from build123d import *

# Parameters (mm, degrees)
BOSS_EXTRUDE1_DEPTH        = 8
F_11_0_11_DIAMETER_HOLE5_D = 11


with BuildPart() as part:
    # Sketch1 → Boss-Extrude1 (new body)
    with BuildSketch(Plane.XY):
        with BuildLine():
            Line((20, -75), (-20, -75))
            ThreePointArc((-20, -75), (-23.535533906, -73.535533906), (-25, -70))
            Line((-25, -70), (-25, 70))
            ThreePointArc((-25, 70), (-23.535533906, 73.535533906), (-20, 75))
            Line((-20, 75), (20, 75))
            ThreePointArc((20, 75), (23.535533906, 73.535533906), (25, 70))
            Line((25, 70), (25, -70))
            ThreePointArc((25, -70), (23.535533906, -73.535533906), (20, -75))
        make_face()
    extrude(amount=BOSS_EXTRUDE1_DEPTH)

    # Ø11.0 (11) Diameter Hole5 (through all)
    with Locations(Plane.XY.offset(8)):
        with Locations((0, 52.5), (0, -52.5)):
            Hole(F_11_0_11_DIAMETER_HOLE5_D / 2)


solid = part.part
Here's how the part is built. I have some questions about the finished solid (model axes, mm). Coordinates: 2 decimals unless noted, no trailing zeros. Order: outer loops, then holes, each group sorted by start corner. A loop starts at its lowest first (then second) coordinate and runs counter-clockwise, first axis right, second up.
Item 1: If we section it at C-C on z = 2.25: List the corners of the cut face in (x, y) for me.
Result sheet:
outline: (-25, -70) arc R5 ccw to (-20, -75) - (20, -75) arc R5 ccw to (25, -70) - (25, 70) arc R5 ccw to (20, 75) - (-20, 75) arc R5 ccw to (-25, 70) - close; hole circle Ø11 at (0, -52.5); hole circle Ø11 at (0, 52.5)
Item 2: For P1, Ø6.5, axis at x = 0, y = -52.5, coming from the -Z side; P2, Ø14.5, axis at x = 0, y = 52.5, coming from the -Z side, each with a flat end and sliding along its axis, tell me the tip position at first contact or that it passes through.
Result sheet:
P1: passes through
P2: stops at z = 0
Item 3: If we section it at B-B on y = -52.5: List the corners of the cut face in (x, z) for me, plus the area to 3 significant figures.
Result sheet:
outline: (-25, 0) - (-5.5, 0) - (-5.5, 8) - (-25, 8) - close; (5.5, 0) - (25, 0) - (25, 8) - (5.5, 8) - close
area: 312 mm2
Item 4: If we section it at A-A on x = 0: List the corners of the cut face in (y, z) for me, plus the area to 3 significant figures.
Result sheet:
outline: (-75, 0) - (-58, 0) - (-58, 8) - (-75, 8) - close; (-47, 0) - (47, 0) - (47, 8) - (-47, 8) - close; (58, 0) - (75, 0) - (75, 8) - (58, 8) - close
area: 1,020 mm2
Item 5: If we mould it in two halves opening along Y, with no side actions, what happens to faces 1 (the face through (0, 1, 0)), 2 (the face through (0.716, -47.047, 3.944)), 3 (the face through (0, 75, 4))? For each: +Y half, -Y half, draft (parallel to the pull), parting line (faces both ways), or undercut.
Result sheet:
face 1: draft
face 2: undercut
face 3: +Y half
Item 6: I need wall thicknesses on line 1 (Y direction, x = 0, z = 5.25); line 2 (Y direction, x = -3, z = 2); line 3 (X direction, y = 48.5, z = 6.25). Which ranges of each line are inside material? Lowest first, please.
Result sheet:
line 1: y = -75 to -58, -47 to 47, 58 to 75
line 2: y = -75 to -57.11, -47.89 to 47.89, 57.11 to 75
line 3: x = -25 to -3.77, 3.77 to 25
